Source: three-view drawing plus pictorial views. Frame: mm from the lowest corner of the part. A direction names the side the tool comes from. Round coordinates to 2 decimals unless told otherwise and drop trailing zeros. Loops run counter-clockwise (first coordinate to the right, second up) from the corner with the lowest first, then second, coordinate; pieces in that order, holes last. Notation, with made-up numbers: M 66,6 L 71,6 A29 ccw 71,45 Z; hole C 75.5,8 d11. An arc over 180 degrees is marked long. Answer as a JSON object with one key per item and string values.
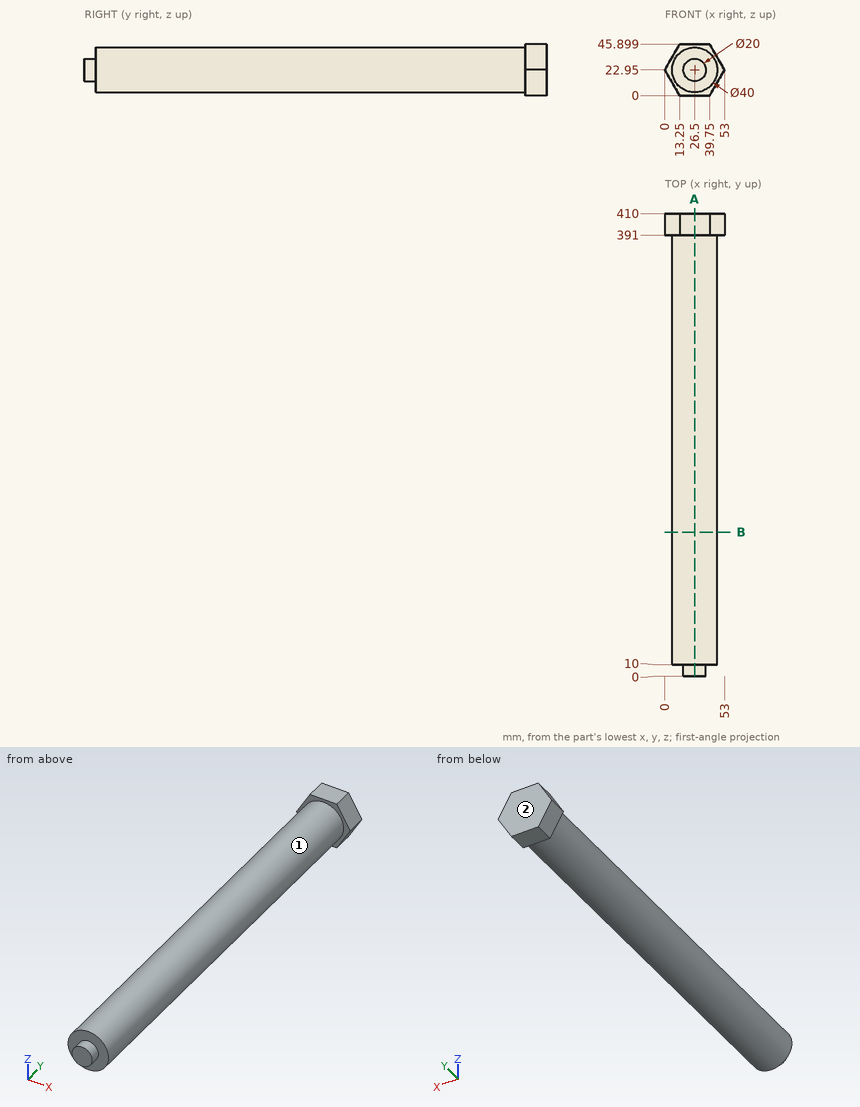
1) Cut plane A-A on x = 26.5. Return the cut outline in (y, z), and give its area (3 significant figures).
Geometry results:
{"outline": "M 0,12.95 L 10,12.95 L 10,2.95 L 391,2.95 L 391,0 L 410,0 L 410,45.9 L 391,45.9 L 391,42.95 L 10,42.95 L 10,32.95 L 0,32.95 Z", "area": "16,300 mm2"}
2) Set-up query: the marked faces 1 and 2. Return all of +Z, -Z, +X, -X, +Y, -Y with unobstructed straight access to the full face (end or side cutting, diameter ignored); none if empty.
Geometry results:
{"face 1": "-Y", "face 2": "+Z, -Z, +X, -X, +Y"}
3) First-contact query: pin 1 (4 mm diameter, centred on x = 44.5, y = 103, fed in from -Z); pin 2 (8 mm diameter, centred on y = 54, z = 30, fed in from -X); pin 3 (4 mm diameter, centred on y = 192, z = 35.5, fed in from -X). Flat tips, straight axial feed; report the tip coordinate or a pass-through.
Geometry results:
{"pin 1": "z = 10.95", "pin 2": "x = 6.73", "pin 3": "x = 9.51"}
4) Cut plane B-B on y = 127.5. Return the cut outline in (x, z), and give its area (3 significant figures).
Geometry results:
{"outline": "C 26.5,22.95 d40", "area": "1,260 mm2"}
5) Line query: probe 1 along Y at (x, z) = (29.5, 12.5); probe 2 along Y at (x, z) = (13, 6.5); probe 3 along X at (y, z) = (243, 8) (1 decimal). Output: solid intervals per line, ascending.
Geometry results:
{"probe 1": "10 to 410", "probe 2": "391 to 410", "probe 3": "13.2 to 39.8"}
